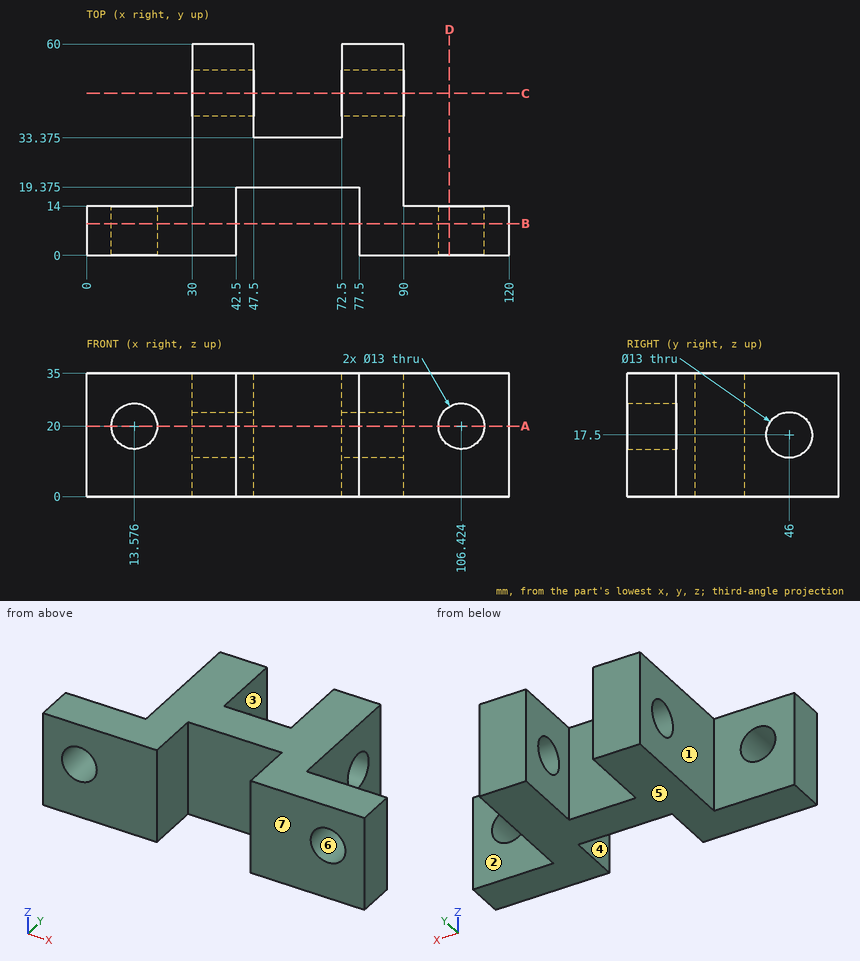
Answer from the drawing. Dimensions are ordinates in mm from the lowest x, y and z of the part. A direction names the side the tool comes from. Give positions to 0.01 mm unless a question says otherwise; leave off trailing zeros. Loops run counter-clockwise (first coordinate to the right, second up) from the corner with the lowest first, then second, coordinate; pieces in that order, holes last.
Item 1: A cutting plane is placed at B-B (y = 9). Give the vertices of the cut face in (x, z).
Derived:
outline: (0, 0) - (42.5, 0) - (42.5, 35) - (0, 35) - close; (77.5, 0) - (120, 0) - (120, 35) - (77.5, 35) - close; hole circle Ø13 at (13.58, 20); hole circle Ø13 at (106.42, 20)
Item 2: A tool of negligible diameter and unlimited length cuts with its end or side. For the marked faces 1, 2, 3 and 4, from which of +Z, -Z, +X, -X, +Y, -Y can it reach the whole face along a straight path? Write none if from no direction.
Derived:
face 1: +Z, -Z, -X, +Y
face 2: +Z, -Z, +X, +Y
face 3: +Z, -Z, +Y
face 4: +Z, -Z, -Y
Item 3: A cutting plane is placed at C-C (y = 46). Give the vertices of the cut face in (x, z).
Derived:
outline: (30, 0) - (47.5, 0) - (47.5, 11) - (30, 11) - close; (30, 24) - (47.5, 24) - (47.5, 35) - (30, 35) - close; (72.5, 0) - (90, 0) - (90, 11) - (72.5, 11) - close; (72.5, 24) - (90, 24) - (90, 35) - (72.5, 35) - close
Item 4: A cutting plane is placed at A-A (z = 20). Give the number of separate pieces and of enclosed holes in the cut face, then the cut area to 3 significant figures.
Derived:
separate pieces: 5
enclosed holes: 0
area: 2,310 mm2
Item 5: Each of these flat-tipped pins is pushed along its axis until it touches: pin 1 Ø8 at (y, z) = (53, 23) entering from -X; pin 2 Ø10.5 at (x, z) = (13.58, 20) entering from +Y; pin 3 Ø1.5 at (x, y) = (21, 7.5) entering from -Z; pin 4 Ø7.5 at (x, z) = (60, 17.5) entering from +Y (1 decimal). Where does it stop, or does it pass through?
Derived:
pin 1: stops at x = 30
pin 2: passes through
pin 3: stops at z = 0
pin 4: stops at y = 33.4
Item 6: A cutting plane is placed at D-D (x = 103). Give the vertices of the cut face in (y, z) (1 decimal).
Derived:
outline: (0, 0) - (14, 0) - (14, 14.5) - (0, 14.5) - close; (0, 25.5) - (14, 25.5) - (14, 35) - (0, 35) - close
Item 7: Determine the mould class of the marked faces 5, 6 and 7 for opening direction Z: +Z half, -Z half, draft (parallel to the pull), parting line (faces both ways), or undercut.
Derived:
face 5: -Z half
face 6: undercut
face 7: draft
Item 8: Find the intervals of material crossed by line 1 along Y through (x, z) = (36, 17.5); line 2 along X through (y, z) = (41, 30); line 3 along X through (y, z) = (6.5, 24.5) (1 decimal), in increasing order.
Derived:
line 1: y = 0 to 39.5, 52.5 to 60
line 2: x = 30 to 47.5, 72.5 to 90
line 3: x = 0 to 8.9, 18.3 to 42.5, 77.5 to 101.7, 111.1 to 120
